```python
from build123d import *

# Parameters (mm, degrees)
CUT_EXTRUDE1_DEPTH      = 10
CUT_EXTRUDE1_DEPTH_BACK = 59.532042507
SKETCH2_R               = 3
SKETCH2_R_2             = 1.5
SKETCH2_R_3             = 2
CHAMFER1_SIZE           = 1
CHAMFER2_SIZE           = 2


with BuildPart() as part:
    # Sketch1 → Revolve1 (revolve)
    with BuildSketch(Plane(origin=(0, 0, 0), x_dir=(0, 0, -1), z_dir=(1, 0, 0)), mode=Mode.PRIVATE) as revolve1_sk:
        Polygon((0, 0), (0, 24), (-2, 24), (-2, 41), (-10, 41), (-10, 0), align=None)
    revolve(revolve1_sk.sketch.rotate(Axis((0, 0, 25.9375), (0, 0, -1)), 90), axis=Axis((0, 0, 25.9375), (0, 0, -1)))

    # Sketch2 → Cut-Extrude1 (cut, two sides: drawn at the far end of the back side and taken through both)
    with BuildSketch(Plane(origin=(0, 0, 2), x_dir=(-1, 0, 0), z_dir=(0, 0, -1)).offset(-CUT_EXTRUDE1_DEPTH_BACK)):
        with Locations(Location((0, 35, 0), (0, 0, 180))):
            Circle(SKETCH2_R)
        with Locations(Location((30.310889132, 17.5, 0), (0, 0, 180))):
            Circle(SKETCH2_R)
        with Locations(Location((30.310889132, -17.5, 0), (0, 0, 180))):
            Circle(SKETCH2_R)
        with Locations(Location((0, -35, 0), (0, 0, 180))):
            Circle(SKETCH2_R)
        with Locations(Location((-30.310889132, -17.5, 0), (0, 0, 180))):
            Circle(SKETCH2_R)
        with Locations(Location((-30.310889132, 17.5, 0), (0, 0, 180))):
            Circle(SKETCH2_R)
        with Locations(Location((17.5, -30.310889132, 0), (0, 0, 180))):
            Circle(SKETCH2_R_2)
        with Locations(Location((0, 5, 0), (0, 0, 180))):
            Circle(SKETCH2_R_3)
    extrude(amount=CUT_EXTRUDE1_DEPTH + CUT_EXTRUDE1_DEPTH_BACK, mode=Mode.SUBTRACT)

    # Chamfer1
    chamfer1_edges = [part.edges().sort_by_distance(p)[0] for p in [
        (-41, 0, 10),
    ]]
    chamfer(chamfer1_edges, length=CHAMFER1_SIZE)

    # Chamfer2
    chamfer2_edges = [part.edges().sort_by_distance(p)[0] for p in [
        (-2, 5, 10),
    ]]
    chamfer(chamfer2_edges, length=CHAMFER2_SIZE)


solid = part.part
```
Could you check a few things on this model? Use its own coordinates, in mm. A direction names the side the tool comes from. Round coordinates to 2 decimals unless told otherwise and drop trailing zeros. Write each loop counter-clockwise with the first axis right and the second up, starting at its lowest first coordinate (ties: lowest second). Pieces come first, ordered by that corner, then holes.
(1) Which directions (+Z, -Z, +X, -X, +Y, -Y) give clear straight access to the entire face, cutting with the end or side of a thin tool? Please do faces 4 (the face through (-17.825, -28.847, 6.056)), 5 (the face through (-18, 18, 2)).
Findings below:
face 4: +Z, -Z
face 5: -Z
(2) Thinking about a two-plate mould opening in X: for faces 1 (the face through (22.89, -7.21, 1.01)), 2 (the face through (0, -38, 6)), 3 (the face through (-1, -1, 10)), which applies, +X half, -X half, draft (parallel to the pull), parting line (faces both ways), or undercut?
Findings below:
face 1: parting line
face 2: undercut
face 3: draft
(3) Suppose I cut it at C-C on z = 5.25. State how many separate pieces and enclosed holes the cut face has, and give its area (3 significant figures).
Findings below:
separate pieces: 1
enclosed holes: 8
area: 5,090 mm2
(4) For pin 1 (4 mm diameter, centred on x = -5, z = 4.5, fed in from +Y); pin 2 (8 mm diameter, centred on x = -30.31, y = -17.5, fed in from -Z); pin 3 (5 mm diameter, centred on y = -10, z = 2, fed in from +X), each with a flat end and sliding along its axis, tell me the tip position at first contact or that it passes through.
Findings below:
pin 1: stops at y = 40.89
pin 2: stops at z = 2
pin 3: stops at x = 40.31
(5) Suppose I cut it at A-A on x = 0. Write out the boundary of the cut face in (y, z), and give its area (3 significant figures).
Findings below:
outline: (-41, 2) - (-38, 2) - (-38, 10) - (-40, 10) - (-41, 9) - close; (-32, 2) - (-24, 2) - (-24, 0) - (3, 0) - (3, 8) - (1, 10) - (-32, 10) - close; (7, 0) - (24, 0) - (24, 2) - (32, 2) - (32, 10) - (9, 10) - (7, 8) - close; (38, 2) - (41, 2) - (41, 9) - (40, 10) - (38, 10) - close
area: 611 mm2
(6) If I drill on probe 1 along X at (y, z) = (-17, 9.25); probe 2 along Y at (x, z) = (-33, 4.75); probe 3 along Y at (x, z) = (-17.5, 5.25), over which ranges is the centre line in solid material (lowest first)?
Findings below:
probe 1: x = -37.03 to -33.27, -27.35 to 27.35, 33.27 to 37.03
probe 2: y = -24.33 to -18.83, -16.17 to 16.17, 18.83 to 24.33
probe 3: y = -37.08 to -31.81, -28.81 to 37.08
(7) Suppose I cut it at B-B on y = 0. Write out the boundary of the cut face in (x, z), and give its area (3 significant figures).
Findings below:
outline: (-41, 2) - (-24, 2) - (-24, 0) - (24, 0) - (24, 2) - (41, 2) - (41, 9) - (40, 10) - (-40, 10) - (-41, 9) - close
area: 751 mm2
